The listing builds one solid part. Answer for the finished solid, in the listing's coordinates (mm). Face numbers are marked on the shaded views. A direction names the side the tool comes from. Coordinates: 2 decimals unless noted, no trailing zeros. Order: outer loops, then holes, each group sorted by start corner. A loop starts at its lowest first (then second) coordinate and runs counter-clockwise, first axis right, second up. Notation, with made-up numbers: M -33,-39.75 L 19,-39.75 A20 ccw 19,-9.75 Z; hole C -2.5,72 d7. An arc over 180 degrees is marked long. One line per item, written item: value. Start each with the question number.
Q1. The part is cut by section C-C on z = 8. Give the vertices of the cut face in (x, y), then the cut area to 3 significant figures.
Q2. For the marked faces 4 and 5, determine the directions among +Z, -Z, +X, -X, +Y, -Y from which every point of the face is accessible in a straight line to the end or side of a thin tool.
Q3. Each of these flat-tipped pins is pushed along its axis until it touches: pin 1 Ø5 at (y, z) = (0.5, 4.5) entering from +X; pin 2 Ø6 at (x, y) = (4.5, 4) entering from -Z; pin 3 Ø1.5 at (x, z) = (3.5, -1) entering from -Y; pin 4 Ø5 at (x, z) = (-4, 20) entering from -Y. Where does it stop, or does it pass through?
Q4. Determine the mould class of the marked faces 1, 2 and 3 for opening direction Z: pulls with the +Z half, pulls with the -Z half, needs draft (parallel to the pull), parting line crosses it, or undercut.
Q5. The part is cut by section D-D on z = 20.5. Give the vertices of the cut face in (x, y), then the cut area to 3 significant figures.
Q6. The part is cut by section A-A on y = 0. Give the vertices of the cut face in (x, z), then the cut area to 3 significant figures.
Q7. Straight lines are drawn through the part: line 1 along Z through (x, y) = (-3, 4); line 2 along Z through (x, y) = (2, -5); line 3 along Y through (x, z) = (5, 19.5). For each, find the intervals that lie inside material, in ascending order. Write a range as [from, to].
```python
from build123d import *

# Parameters (mm, degrees)
SKETCH_1_R      = 3
EXTRUDE_1_DEPTH = 19
SKETCH_2_R      = 6
EXTRUDE_2_DEPTH = 4
CHAMFER_1_SIZE  = 1
EXTRUDE_START   = 4
SKETCH_3_R      = 6
EXTRUDE_3_DEPTH = 4
CHAMFER_2_SIZE  = 1


with BuildPart() as part:
    # 草图1 → 凸台-拉伸1 (new body)
    with BuildSketch(Plane.XY):
        Circle(SKETCH_1_R)
    extrude(amount=EXTRUDE_1_DEPTH)

    # 草图2 → 凸台-拉伸2 (add)
    with BuildSketch(Plane.XY.offset(19)):
        Circle(SKETCH_2_R)
    extrude(amount=EXTRUDE_2_DEPTH)

    # 倒角1
    chamfer_1_edges = [part.edges().sort_by_distance(p)[0] for p in [
        (-6, 0, 23),
    ]]
    chamfer(chamfer_1_edges, length=CHAMFER_1_SIZE)

    # 草图3 → 凸台-拉伸3 (add)
    with BuildSketch(Plane(origin=(0, 0, 0), x_dir=(-1, 0, 0), z_dir=(0, 0, -1)).offset(EXTRUDE_START)):
        with Locations(Location((0, 0, 0), (0, 0, 180))):
            Circle(SKETCH_3_R)
    extrude(amount=-EXTRUDE_3_DEPTH)

    # 倒角2
    chamfer_2_edges = [part.edges().sort_by_distance(p)[0] for p in [
        (-6, 0, -4),
    ]]
    chamfer(chamfer_2_edges, length=CHAMFER_2_SIZE)


solid = part.part
```
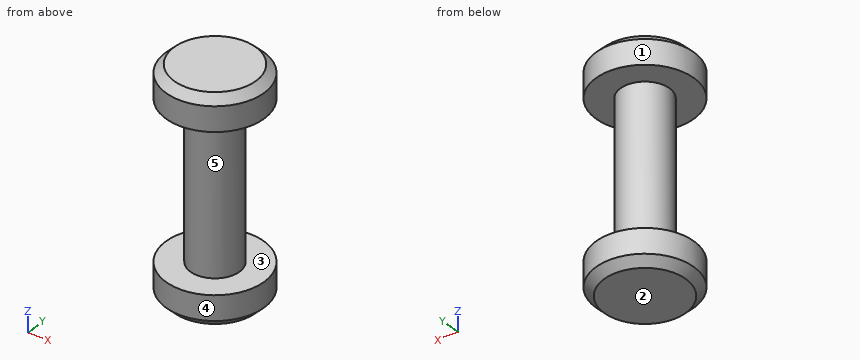
Output:
1. outline: C 0,0 d6
1. area: 28.3 mm^2
2. face 4: +Z, -Z
2. face 5: none
3. pin 1: stops at x = 3
3. pin 2: stops at z = -4
3. pin 3: stops at y = -5.33
3. pin 4: stops at y = -5.81
4. face 1: needs draft
4. face 2: pulls with the -Z half
4. face 3: undercut
5. outline: C 0,0 d12
5. area: 113 mm^2
6. outline: M -6,-3 L -5,-4 L 5,-4 L 6,-3 L 6,0 L 3,0 L 3,19 L 6,19 L 6,22 L 5,23 L -5,23 L -6,22 L -6,19 L -3,19 L -3,0 L -6,0 Z
6. area: 208 mm^2
7. line 1: z = [-4, 0], [19, 23]
7. line 2: z = [-3.61, 0], [19, 22.61]
7. line 3: y = [-3.32, 3.32]
